from build123d import *

# Parameters (mm, degrees)
SKETCH_1_W                = 190
SKETCH_1_H                = 70
EXTRUDE_1_DEPTH           = 15
CHAMFER_1_SIZE            = 3
HOLE_WIZARD_5_D           = 6.6
HOLE_WIZARD_5_CBORE_D     = 11
HOLE_WIZARD_5_CBORE_DEPTH = 6.8
HOLE_WIZARD_3_D           = 9
HOLE_WIZARD_3_CBORE_D     = 15
HOLE_WIZARD_3_CBORE_DEPTH = 9
HOLE_WIZARD_M8_1_D        = 6.8


with BuildPart() as part:
    # 草图1 → 凸台-拉伸1 (new body)
    with BuildSketch(Plane(origin=(0, 0, 0), x_dir=(1, 0, 0), z_dir=(0, 1, 0))):
        Rectangle(SKETCH_1_W, SKETCH_1_H)
    extrude(amount=EXTRUDE_1_DEPTH)

    # 倒角1
    chamfer_1_edges = [part.edges().sort_by_distance(p)[0] for p in [
        (95, 7.5, 35),
        (-95, 7.5, 35),
        (-95, 7.5, -35),
        (95, 7.5, -35),
    ]]
    chamfer(chamfer_1_edges, length=CHAMFER_1_SIZE)

    # 打孔尺寸(%根据)内六角圆柱头螺钉的类型5 (through all)
    with Locations(Plane(origin=(0, 15, 0), x_dir=(1, 0, 0), z_dir=(0, 1, 0))):
        with Locations((75, -26), (25, -26), (-25, -26), (-75, -26), (25, 26), (-25, 26), (-75, 26), (75, 26)):
            CounterBoreHole(HOLE_WIZARD_5_D / 2, HOLE_WIZARD_5_CBORE_D / 2, HOLE_WIZARD_5_CBORE_DEPTH)

    # 打孔尺寸(%根据)内六角圆柱头螺钉的类型3 (through all)
    with Locations(Plane(origin=(0, 0, 0), x_dir=(-1, 0, 0), z_dir=(0, -1, 0))):
        with Locations((35, 0), (75, 0)):
            CounterBoreHole(HOLE_WIZARD_3_D / 2, HOLE_WIZARD_3_CBORE_D / 2, HOLE_WIZARD_3_CBORE_DEPTH)

    # M8 螺纹孔1 (through all)
    with Locations(Plane(origin=(0, 15, 0), x_dir=(1, 0, 0), z_dir=(0, 1, 0))):
        with Locations((55, 0), (35, 0)):
            Hole(HOLE_WIZARD_M8_1_D / 2)


solid = part.part
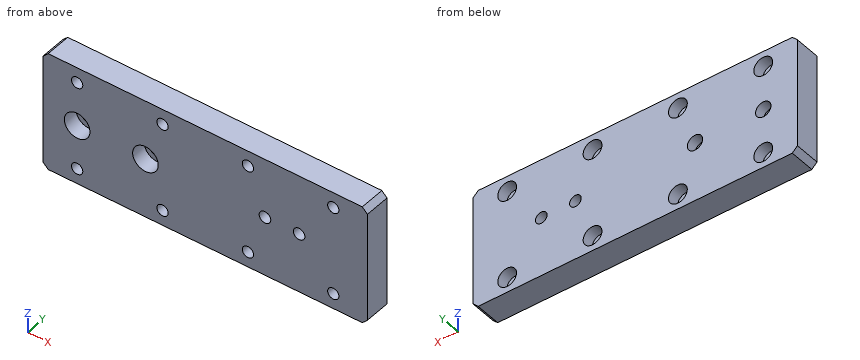
Model file for the job. Use its own axes, mm. Coordinates: 2 decimals unless noted, no trailing zeros. Write each loop counter-clockwise with the first axis right and the second up, starting at its lowest first coordinate (ties: lowest second). Pieces come first, ordered by that corner, then holes. Notation, with made-up numbers: (-32, 46.5) - (13, 46.5) arc R19 ccw to (13, 51.5) - close; hole circle Ø8 at (12.25, 48). An arc over 180 degrees is marked (long way). Write each question's results on one line, items separated by ' | '. Start each with the question number.
1) Cut at A-A (z = 0). Write the cut outline in (x, y).
2) Probe line 1 along X through (y, z) = (2.25, 26); line 2 along Z through (x, y) = (25, 5.25); line 3 along X through (y, z) = (13, -26). List the from-to ranges inside material, lowest first. Write a range as from..to.
3) Cut at C-C (x = 35). Write the cut outline in (y, z).
4) Flat gauge pins, fed straight in: P1, Ø10.5, axis at x = -75, z = -26, coming from the +Y side; P2, Ø7.5, axis at x = -33, z = -2.5, coming from the -Y side. Where does each tip first touch, or does it go through?
5) Cut at D-D (x = -75). Write the cut outline in (y, z).
6) Cut at B-B (y = 1.75). Count the separate pieces of the cut face and the enclosed holes in it, then the cut area to 3 significant figures.
Returned:
1) outline: (-95, 0) - (-82.5, 0) - (-82.5, 9) - (-79.5, 9) - (-79.5, 15) - (-95, 15) - close; (-70.5, 9) - (-67.5, 9) - (-67.5, 0) - (-42.5, 0) - (-42.5, 9) - (-39.5, 9) - (-39.5, 15) - (-70.5, 15) - close; (-30.5, 9) - (-27.5, 9) - (-27.5, 0) - (31.6, 0) - (31.6, 15) - (-30.5, 15) - close; (38.4, 0) - (51.6, 0) - (51.6, 15) - (38.4, 15) - close; (58.4, 0) - (95, 0) - (95, 15) - (58.4, 15) - close
2) line 1: -95..-78.3, -71.7..-28.3, -21.7..21.7, 28.3..71.7, 78.3..95 | line 2: -35..-29.3, -22.7..22.7, 29.3..35 | line 3: -95..-80.5, -69.5..-30.5, -19.5..19.5, 30.5..69.5, 80.5..95
3) outline: (0, -35) - (15, -35) - (15, -3.4) - (0, -3.4) - close; (0, 3.4) - (15, 3.4) - (15, 35) - (0, 35) - close
4) P1: y = 8.2 | P2: y = 9
5) outline: (0, -35) - (15, -35) - (15, -31.5) - (8.2, -31.5) - (8.2, -29.3) - (0, -29.3) - close; (0, -22.7) - (8.2, -22.7) - (8.2, -20.5) - (15, -20.5) - (15, -4.5) - (9, -4.5) - (9, -7.5) - (0, -7.5) - close; (0, 7.5) - (9, 7.5) - (9, 4.5) - (15, 4.5) - (15, 20.5) - (8.2, 20.5) - (8.2, 22.7) - (0, 22.7) - close; (0, 29.3) - (8.2, 29.3) - (8.2, 31.5) - (15, 31.5) - (15, 35) - (0, 35) - close
6) separate pieces: 1 | enclosed holes: 12 | area: 12,600 mm^2
